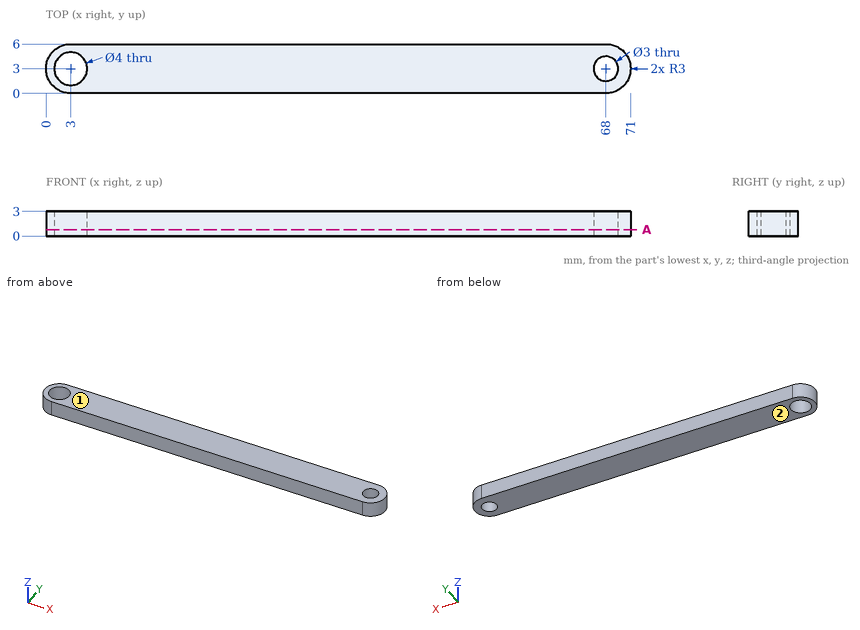
Geometry: see drawing. Coordinates: mm, zero at the bounding-box minimum. Round coordinates to 2 decimals unless told otherwise and drop trailing zeros. Loops run counter-clockwise (first coordinate to the right, second up) from the corner with the lowest first, then second, coordinate; pieces in that order, holes last. Notation, with made-up numbers: (35.25, 53.5) -> (66.25, 53.5) arc R24 cw to (66.25, 65.5) -> close; hole circle Ø1 at (-35.5, 86). An arc over 180 degrees is marked (long way). Write each question's results on one line, items separated by ' | '.
Item 1: Line query: probe 1 along Y at (x, z) = (3, 2.1); probe 2 along Y at (x, z) = (68, 2); probe 3 along X at (y, z) = (2.6, 1.2). Output: solid intervals per line, ascending. Write a range as [from, to].
Answers below:
probe 1: y = [0, 1], [5, 6] | probe 2: y = [0, 1.5], [4.5, 6] | probe 3: x = [0.03, 1.04], [4.96, 66.55], [69.45, 70.97]
Item 2: Pin query (flat end, axial travel): pin 1 Ø1 at (y, z) = (2, 2) entering from +X. Return the tip coordinate at first contact, or that it passes through.
Answers below:
pin 1: stops at x = 70.96
Item 3: Cut plane A-A on z = 0.8. Return the cut outline in (x, y).
Answers below:
outline: (3, 0) -> (68, 0) arc R3 ccw to (68, 6) -> (3, 6) arc R3 ccw to start; hole circle Ø4 at (3, 3); hole circle Ø3 at (68, 3)
Item 4: Pull-direction query (Z, two-part tool) for the marked faces 1 and 2; classes: pulls with the +Z half, pulls with the -Z half, needs draft (parallel to the pull), parting line crosses it, or undercut.
Answers below:
face 1: pulls with the +Z half | face 2: pulls with the -Z half
